The listing builds one solid part. Answer for the finished solid, in the listing's coordinates (mm). Face numbers are marked on the shaded views. A direction names the side the tool comes from. Coordinates: 2 decimals unless noted, no trailing zeros. Order: outer loops, then holes, each group sorted by start corner. A loop starts at its lowest first (then second) coordinate and runs counter-clockwise, first axis right, second up. Notation, with made-up numbers: (63, -12.75) -> (84, -12.75) arc R31 cw to (84, 25.25) -> close; hole circle Ø8 at (30.5, -12). An arc over 180 degrees is marked (long way). Write item = value, one per line. Start each with the question number.
```python
from build123d import *

# Parameters (mm, degrees)
SKETCH6_R           = 6
BOSS_EXTRUDE1_DEPTH = 14
CHAMFER1_SIZE       = 0.5
SKETCH7_W           = 15
SKETCH7_H           = 1
CUT_EXTRUDE1_DEPTH  = 10


with BuildPart() as part:
    # Sketch1 → Revolve1 (revolve)
    with BuildSketch(Plane.XY, mode=Mode.PRIVATE) as revolve1_sk:
        Polygon((0, 0), (0, 10), (191, 10), (191, 6), (256, 6), (256, 0), align=None)
    revolve(revolve1_sk.sketch.rotate(Axis((0, 0, 0), (1, 0, 0)), 90), axis=Axis((0, 0, 0), (1, 0, 0)))

    # Sketch6 → Boss-Extrude1 (add)
    with BuildSketch(Plane.ZY):
        Circle(SKETCH6_R)
    extrude(amount=BOSS_EXTRUDE1_DEPTH)

    # Chamfer1
    chamfer1_edges = [part.edges().sort_by_distance(p)[0] for p in [
        (-14, 0, -6),
    ]]
    chamfer(chamfer1_edges, length=CHAMFER1_SIZE)

    # Sketch7 → Cut-Extrude1 (cut, symmetric)
    with BuildSketch(Plane.XY):
        with Locations((183.5, 9.5)):
            Rectangle(SKETCH7_W, SKETCH7_H)
        with Locations((183.5, -9.5)):
            Rectangle(SKETCH7_W, SKETCH7_H)
    extrude(amount=CUT_EXTRUDE1_DEPTH, both=True, mode=Mode.SUBTRACT)


solid = part.part
```
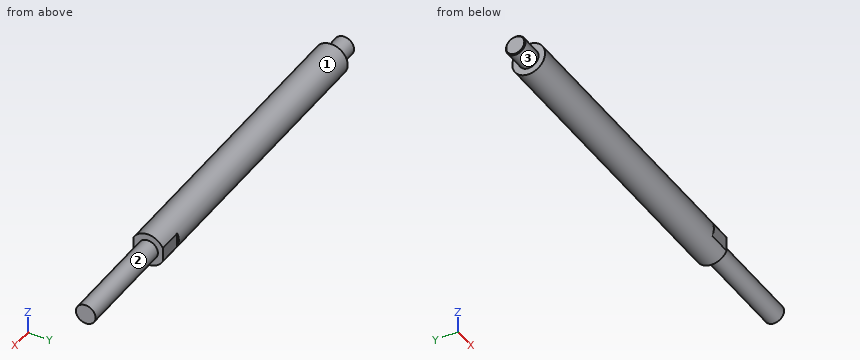
Item 1: Each of these flat-tipped pins is pushed along its axis until it touches: pin 1 (2 mm diameter, centred on y = -7.5, z = -5, fed in from +X); pin 2 (0.8 mm diameter, centred on y = 9.5, z = 1.5, fed in from +X); pin 3 (5 mm diameter, centred on x = 126.5, y = -6, fed in from +Z). Where does it stop, or does it pass through?
Item 2: Section A-A, the plane y = 0 is taken. Give the vertices of the cut face in (x, z), then the cut area to 3 significant figures.
Item 3: Consider probe 1 along X at (y, z) = (-2, -5.75); probe 2 along Z at (x, y) = (146, 1); probe 3 along Y at (x, z) = (209, 0.75). Determine where each line is inside the solid, lowest interval first.
Item 4: Section D-D, the plane x = 143 is taken. Give the vertices of the cut face in (y, z).
Item 5: Which of the six approach directions +Z, -Z, +X, -X, +Y, -Y give full straight-line access (tool end or side, diameter ignored) to the marked faces 1, 2 and 3?
Item 6: Section B-B, the plane z = 0 is taken. Give the vertices of the cut face in (x, y).
Item 7: Section C-C, the plane x = 186 is taken. Give the vertices of the cut face in (y, z), then the cut area to 3 significant figures.
A:
q1.pin_1 = 191
q1.pin_2 = 176
q1.pin_3 = 9.37
q2.outline = (-14, -5.5) -> (-13.5, -6) -> (0, -6) -> (0, -10) -> (191, -10) -> (191, -6) -> (256, -6) -> (256, 6) -> (191, 6) -> (191, 10) -> (0, 10) -> (0, 6) -> (-13.5, 6) -> (-14, 5.5) -> close
q2.area = 4,770 mm^2
q3.probe_1 = 0 to 191
q3.probe_2 = -9.95 to 9.95
q3.probe_3 = -5.95 to 5.95
q4.outline = circle Ø20 at (0, 0)
q5.face_1 = +X, -X
q5.face_2 = +X
q5.face_3 = -X
q6.outline = (-14, -5.5) -> (-13.5, -6) -> (0, -6) -> (0, -10) -> (176, -10) -> (176, -9) -> (191, -9) -> (191, -6) -> (256, -6) -> (256, 6) -> (191, 6) -> (191, 9) -> (176, 9) -> (176, 10) -> (0, 10) -> (0, 6) -> (-13.5, 6) -> (-14, 5.5) -> close
q7.outline = (-9, -4.36) arc R10 ccw to (9, -4.36) -> (9, 4.36) arc R10 ccw to (-9, 4.36) -> close
q7.area = 302 mm^2
